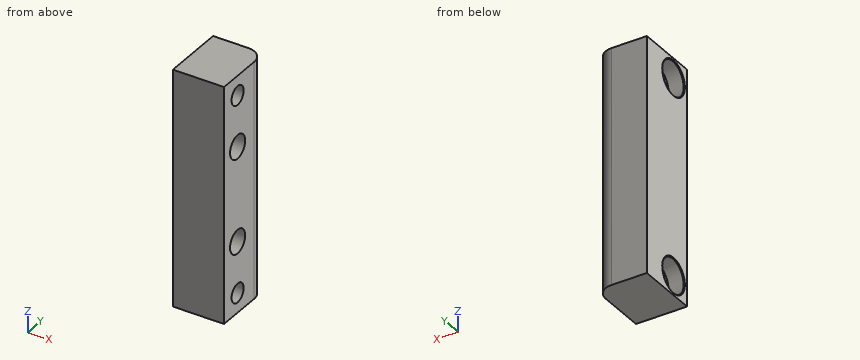
from build123d import *

# Parameters (mm, degrees)
SKETCH_1_W                   = 30
SKETCH_1_H                   = 8
EXTRUDE_1_DEPTH              = 6.5
HOLE_WIZARD_3_0_3_1_D        = 3
HOLE_WIZARD_3_0_3_1_DEPTH    = 3
HOLE_WIZARD_M2_1_D           = 2.4
HOLE_WIZARD_M2_1_CBORE_D     = 4.3
HOLE_WIZARD_M2_1_CBORE_DEPTH = 2
CHAMFER_1_SIZE               = 0.1
CHAMFER_1_SIZE2              = 0.096568877
FILLET_1_R                   = 2


with BuildPart() as part:
    # 草图1 → 凸台-拉伸1 (new body)
    with BuildSketch(Plane(origin=(3.25, 0, 0), x_dir=(0, 0, -1), z_dir=(1, 0, 0))):
        with Locations((-15, 0)):
            Rectangle(SKETCH_1_W, SKETCH_1_H)
    extrude(amount=-EXTRUDE_1_DEPTH)

    # Ø3.0 (3) 直径孔1
    with Locations(Plane(origin=(3.25, 0, 0), x_dir=(0, 0, -1), z_dir=(1, 0, 0))):
        with Locations((-9, -1.3), (-21, -1.3)):
            Hole(HOLE_WIZARD_3_0_3_1_D / 2, depth=HOLE_WIZARD_3_0_3_1_DEPTH)

    # M2 六角头机械螺钉的柱形沉头孔1 (through all)
    with Locations(Plane.ZY.offset(3.25)):
        with Locations((27.5, -1.3), (2.5, -1.3)):
            CounterBoreHole(HOLE_WIZARD_M2_1_D / 2, HOLE_WIZARD_M2_1_CBORE_D / 2, HOLE_WIZARD_M2_1_CBORE_DEPTH)

    # 倒角1
    chamfer_1_edges = [part.edges().sort_by_distance(p)[0] for p in [
        (-3.25, -1.3, 0.35),
        (-3.25, -1.3, 25.35),
    ]]
    chamfer_1_side = [part.faces().sort_by_distance(p)[0] for p in [
        (-3.25, 0.178981568, 15),
    ]]
    chamfer(chamfer_1_edges, length=CHAMFER_1_SIZE, length2=CHAMFER_1_SIZE2, reference=chamfer_1_side[0])

    # 圆角1
    fillet_1_edges = [part.edges().sort_by_distance(p)[0] for p in [
        (3.25, 4, 15),
    ]]
    fillet(fillet_1_edges, radius=FILLET_1_R)


solid = part.part
Geometry: final body of the model. Coordinates: model frame, mm. Coordinates: 2 decimals unless noted, no trailing zeros. Order: outer loops, then holes, each group sorted by start corner. A loop starts at its lowest first (then second) coordinate and runs counter-clockwise, first axis right, second up.
1) Section B-B (x = 0.75). Return loops of the section in (y, z).
Result sheet:
outline: (-4, 0) - (4, 0) - (4, 30) - (-4, 30) - close; hole circle Ø3 at (-1.3, 9); hole circle Ø3 at (-1.3, 21); hole circle Ø2.4 at (-1.3, 2.5); hole circle Ø2.4 at (-1.3, 27.5)
2) Section D-D (x = -1.75). Return loops of the section in (y, z).
Result sheet:
outline: (-4, 0) - (4, 0) - (4, 30) - (-4, 30) - close; hole circle Ø4.3 at (-1.3, 2.5); hole circle Ø4.3 at (-1.3, 27.5)
3) Section C-C (z = 2.5). Return loops of the section in (x, y), then the cut area to 3 significant figures.
Result sheet:
outline: (-3.25, -4) - (3.25, -4) - (3.25, -2.5) - (-1.25, -2.5) - (-1.25, -3.45) - (-3.15, -3.45) - (-3.25, -3.55) - close; (-3.25, 0.95) - (-3.15, 0.85) - (-1.25, 0.85) - (-1.25, -0.1) - (3.25, -0.1) - (3.25, 2) arc R2 ccw to (1.25, 4) - (-3.25, 4) - close
area: 31.7 mm2
4) Ray query, probe 1 along Z at (x, y) = (0, -1); probe 2 along Y at (x, z) = (-1.7, 2.5); probe 3 along Z at (x, y) = (-2, -2). Return the intervals inside material, ascending.
Result sheet:
probe 1: z = 0 to 1.34, 3.66 to 26.34, 28.66 to 30
probe 2: y = -4 to -3.45, 0.85 to 4
probe 3: z = 0 to 0.47, 4.53 to 25.47, 29.53 to 30
5) Section A-A (y = -1.3). Give the number of separate pieces and of enclosed holes in the cut face, then the cut area to 3 significant figures.
Result sheet:
separate pieces: 3
enclosed holes: 0
area: 138 mm2
6) First-contact query: P1, Ø0.9, axis at y = -1.5, z = 8.5, coming from the +X side. Flat tip, straight axial feed; report the tip coordinate or a pass-through.
Result sheet:
P1: stops at x = 0.25
